For this review, use the dimensioned drawing (mm, ordinates from the lowest corner) and the shaded views. A direction names the side the tool comes from. Give positions to 0.01 mm unless a question says otherwise; leave off trailing zeros. Order: outer loops, then holes, each group sorted by start corner. A loop starts at its lowest first (then second) coordinate and runs counter-clockwise, first axis right, second up. Notation, with made-up numbers: M 67,-32 L 111,-32 A6 ccw 111,-25 Z; hole C 77.5,77 d3. An arc over 180 degrees is marked long. Use CSV: the item, a comma, the result in double quotes. Start each with the question number.
(1) Consider section D-D (x = 32). Write out the cut boundary in (y, z).
(2) Draft analysis for pull direction Y (two halves, no side actions). For the marked faces 3, 4 and 5, state which applies: pulls with the +Y half, pulls with the -Y half, needs draft (parallel to the pull), parting line crosses it, or undercut.
(3) Consider section C-C (y = 3.5). Write out the cut boundary in (x, z).
(4) Consider section B-B (z = 20.75). Write out the cut boundary in (x, y).
(5) Consider section A-A (x = 45). Write out the cut boundary in (y, z).
(6) Wall thickness on L1, parallel to Y at x = 35.5, z = 23.5; L2, parallel to Z at x = 49, y = 9.5; L3, parallel to X at y = 5, z = 15 (1 decimal): over which ranges is each line inside the solid? List them lowest first. Write a range as from..to.
(7) Tool access review of the marked faces 1 and 2: name each direction out of +Z, -Z, +X, -X, +Y, -Y from which nothing blocks a thin tool from reaching the whole face with its end or side.
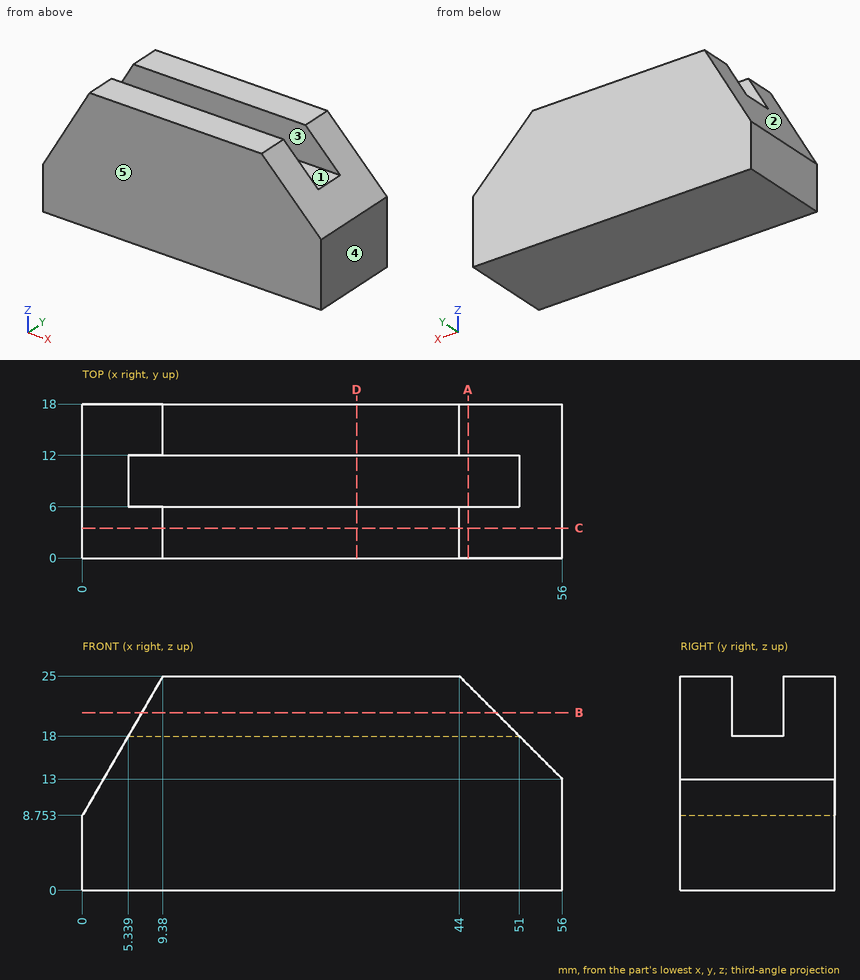
Check result:
1,outline,"M 0,0 L 18,0 L 18,25 L 12,25 L 12,18 L 6,18 L 6,25 L 0,25 Z"
2,face 3,"undercut"
2,face 4,"needs draft"
2,face 5,"pulls with the -Y half"
3,outline,"M 0,0 L 56,0 L 56,13 L 44,25 L 9.38,25 L 0,8.75 Z"
4,outline,"M 6.93,0 L 48.25,0 L 48.25,6 L 6.93,6 Z; M 6.93,12 L 48.25,12 L 48.25,18 L 6.93,18 Z"
5,outline,"M 0,0 L 18,0 L 18,24 L 12,24 L 12,18 L 6,18 L 6,24 L 0,24 Z"
6,L1,"y = 0..6, 12..18"
6,L2,"z = 0..18"
6,L3,"x = 3.6..54"
7,face 1,"+Z, +X, -X"
7,face 2,"+Z, -X, +Y, -Y"
